from build123d import *

# Parameters (mm, degrees)
SKETCH_1_R          = 2
EXTRUDE_1_DEPTH     = 12.5
SKETCH_2_R          = 1.7
CUT_EXTRUDE_1_DEPTH = 21.863604674
CUT_EXTRUDE_2_DEPTH = 6.5


with BuildPart() as part:
    # 草图1 → 凸台-拉伸1 (new, symmetric)
    with BuildSketch(Plane(origin=(0, 0, 0), x_dir=(0, 0, -1), z_dir=(1, 0, 0))):
        with BuildLine():
            Line((0, -3), (-16, -3))
            Line((-16, -3), (-16, -1.8))
            Line((-16, -1.8), (-2.4, -1.8))
            ThreePointArc((-2.4, -1.8), (1.341640786, 2.683281573), (0, -3))
        make_face()
        Circle(SKETCH_1_R, mode=Mode.SUBTRACT)
    extrude(amount=EXTRUDE_1_DEPTH, both=True)

    # 草图2 → 切除-拉伸1 (cut, through all)
    with BuildSketch(Plane(origin=(0, -1.8, 0), x_dir=(1, 0, 0), z_dir=(0, 1, 0))):
        with Locations(Location((-7, -10, 0), (0, 0, 270))):
            Circle(SKETCH_2_R)
        with Locations(Location((7, -10, 0), (0, 0, 270))):
            Circle(SKETCH_2_R)
    extrude(amount=-CUT_EXTRUDE_1_DEPTH, mode=Mode.SUBTRACT)

    # 草图3 → 切除-拉伸2 (cut)
    with BuildSketch(Plane(origin=(12.5, 0, 0), x_dir=(0, 0, -1), z_dir=(1, 0, 0))):
        with BuildLine():
            Line((-4, -3), (0, -3))
            ThreePointArc((0, -3), (1.341640786, 2.683281573), (-2.4, -1.8))
            Line((-2.4, -1.8), (-4, -1.8))
            Line((-4, -1.8), (-4, -3))
        make_face()
    cut_extrude_2 = extrude(amount=-CUT_EXTRUDE_2_DEPTH, mode=Mode.SUBTRACT)

    # 镜向1: 切除-拉伸2 across plane
    add(cut_extrude_2.mirror(Plane(origin=(0, 0, 0), x_dir=(0, 0, 1), z_dir=(1, 0, 0))), mode=Mode.SUBTRACT)


solid = part.part
Geometry check sheet. Reference: the model listing, model coordinates, mm. A direction names the side the tool comes from. Give positions to 0.01 mm unless a question says otherwise; leave off trailing zeros. Write each loop counter-clockwise with the first axis right and the second up, starting at its lowest first coordinate (ties: lowest second). Pieces come first, ordered by that corner, then holes.
1) Cross-section at B-B (y = 0). Record the boundary of the cut face in (x, z).
Values follow:
outline: (-6, -3) - (6, -3) - (6, -2) - (-6, -2) - close; (-6, 2) - (6, 2) - (6, 3) - (-6, 3) - close
2) Go/stop test with flat-tipped pins: pin 1 Ø4 at (x, z) = (-7, 10) entering from +Y; pin 2 Ø1 at (x, y) = (8.5, -2.5) entering from -Z; pin 3 Ø3 at (y, z) = (0, -1) entering from +X. Record where each tip stops, or that it passes through.
Values follow:
pin 1: stops at y = -1.8
pin 2: stops at z = 4
pin 3: stops at x = 6
3) Cross-section at D-D (z = 6.25). Record the boundary of the cut face in (x, y), plus the area to 3 significant figures.
Values follow:
outline: (-12.5, -3) - (12.5, -3) - (12.5, -1.8) - (-12.5, -1.8) - close
area: 30.0 mm2
4) Cross-section at A-A (z = 10). Record the boundary of the cut face in (x, y), plus the area to 3 significant figures.
Values follow:
outline: (-12.5, -3) - (-8.7, -3) - (-8.7, -1.8) - (-12.5, -1.8) - close; (-5.3, -3) - (5.3, -3) - (5.3, -1.8) - (-5.3, -1.8) - close; (8.7, -3) - (12.5, -3) - (12.5, -1.8) - (8.7, -1.8) - close
area: 21.8 mm2
5) Set-up check for faces 4 (the face through (-9, -2, 4)), 5 (the face through (12.5, -2, 10)), 6 (the face through (6, -1, 2)): record each of +Z, -Z, +X, -X, +Y, -Y from which the full face is reachable in a straight line by a thin tool's end or side.
Values follow:
face 4: -Z, -X, +Y, -Y
face 5: +Z, -Z, +X, +Y, -Y
face 6: -Z, +X, +Y, -Y
6) Release check for a two-part mould opening along Y. For faces 1 (the face through (0, -2, 0)), 2 (the face through (-12.5, -2, 10)), 3 (the face through (0, -3, 8)) record: released by +Y, released by -Y, zero draft, split by the parting line, or undercut.
Values follow:
face 1: undercut
face 2: zero draft
face 3: released by -Y
7) Thickness scan on line 1 (X direction, y = -2.35, z = 10); line 2 (Z direction, x = -1, y = 0); line 3 (X direction, y = -2.1, z = 1.5). Record the ranges inside material, lowest first.
Values follow:
line 1: x = -12.5 to -8.7, -5.3 to 5.3, 8.7 to 12.5
line 2: z = -3 to -2, 2 to 3
line 3: x = -6 to 6
8) Cross-section at C-C (x = 7). Record the boundary of the cut face in (y, z), plus the area to 3 significant figures.
Values follow:
outline: (-3, 4) - (-1.8, 4) - (-1.8, 8.3) - (-3, 8.3) - close; (-3, 11.7) - (-1.8, 11.7) - (-1.8, 16) - (-3, 16) - close
area: 10.3 mm2
